Geometry: final body of the model. Coordinates: model frame, mm. Round coordinates to 2 decimals unless told otherwise and drop trailing zeros. Order: outer loops, then holes, each group sorted by start corner. A loop starts at its lowest first (then second) coordinate and runs counter-clockwise, first axis right, second up. Notation, with made-up numbers: M 14,64.5 L 46,64.5 A25 cw 46,101.5 Z; hole C 46.25,-34 d6. An arc over 180 degrees is marked long. Put each result on its own line as item: value. Start each with the question number.
1) Section A-A, the plane z = 15. Return loops of the section in (x, y).
2) Section B-B, the plane x = 13. Return loops of the section in (y, z), then the cut area to 3 significant figures.
3) Material intervals for probe 1 along X at (y, z) = (59, 19); probe 2 along X at (y, z) = (26, 15.75); probe 3 along Y at (x, z) = (86.5, 12.25), sorted ascending. Write a range as [from, to].
4) First-contact query: P1, Ø6, axis at x = 81, z = 6.5, coming from the +Y side; P2, Ø2, axis at x = 43, y = 84, coming from the -Z side; P3, Ø8, axis at y = 49, z = 15, coming from the +X side. Flat tips, straight axial feed; report the tip coordinate or a pass-through.
5) Section C-C, the plane y = 46. Return loops of the section in (x, z), then the cut area to 3 significant figures.
from build123d import *

# Parameters (mm, degrees)
BOSS_EXTRUDE1_DEPTH = 20
CHAMFER1_SIZE       = 15


with BuildPart() as part:
    # Sketch1 → Boss-Extrude1 (new body)
    with BuildSketch(Plane.XY):
        Polygon((0, 0), (100, 0), (100, 25), (25, 100), (0, 100), align=None)
    extrude(amount=BOSS_EXTRUDE1_DEPTH)

    # Chamfer1
    chamfer1_edges = [part.edges().sort_by_distance(p)[0] for p in [
        (0, 0, 10),
    ]]
    chamfer(chamfer1_edges, length=CHAMFER1_SIZE)


solid = part.part
Result sheet:
1. outline: M 0,15 L 15,0 L 100,0 L 100,25 L 25,100 L 0,100 Z
2. outline: M 2,0 L 100,0 L 100,20 L 2,20 Z
2. area: 1,960 mm2
3. probe 1: x = [0, 66]
3. probe 2: x = [0, 99]
3. probe 3: y = [0, 38.5]
4. P1: stops at y = 47
4. P2: passes through
4. P3: stops at x = 80
5. outline: M 0,0 L 79,0 L 79,20 L 0,20 Z
5. area: 1,580 mm2
